The drawing under review shows one solid part. Ordinate dimensions are in mm from its lowest x, y, z. Round coordinates to 2 decimals unless told otherwise and drop trailing zeros. Loops run counter-clockwise (first coordinate to the right, second up) from the corner with the lowest first, then second, coordinate; pieces in that order, holes last. Notation, with made-up numbers: (74.25, 7) -> (128.25, 7) arc R27 cw to (128.25, 36) -> close; hole circle Ø7 at (34, 57). An arc over 180 degrees is marked (long way). Answer as CSV lines item,"result". Start each with the question number.
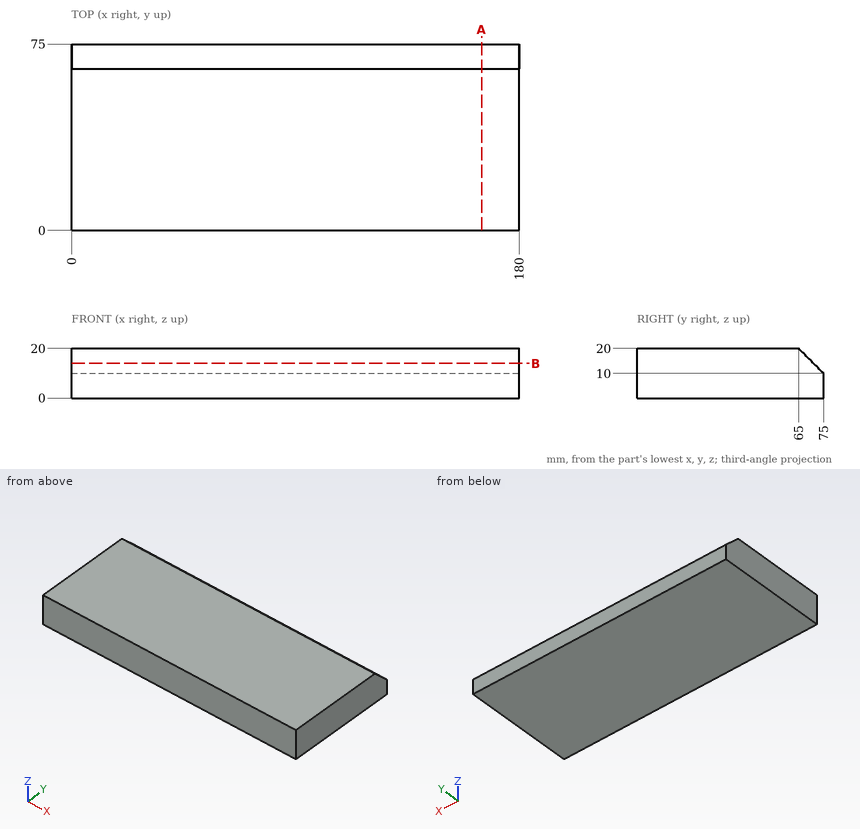
Q1. To check wall thickness, follow probe 1 along Y at (x, z) = (49.5, 18); probe 2 along Y at (x, z) = (75, 13); probe 3 along Z at (x, y) = (140.5, 72.5). State the ranges of each line that lie inside material, in increasing order. Write a range as from..to.
Q2. Add section B-B, the plane z = 14. Give the boundary of the cut face in (x, y), and give its area (3 significant figures).
Q3. Add section A-A, the plane x = 165. Give the boundary of the cut face in (y, z), and give its area (3 significant figures).
Worked answers:
1,probe 1,"y = 0..67"
1,probe 2,"y = 0..72"
1,probe 3,"z = 0..12.5"
2,outline,"(0, 0) -> (180, 0) -> (180, 71) -> (0, 71) -> close"
2,area,"12,800 mm^2"
3,outline,"(0, 0) -> (75, 0) -> (75, 10) -> (65, 20) -> (0, 20) -> close"
3,area,"1,450 mm^2"
